Geometry check sheet. Reference: the model listing, model coordinates, mm. A direction names the side the tool comes from. Give positions to 0.01 mm unless a question says otherwise; leave off trailing zeros. Write each loop counter-clockwise with the first axis right and the second up, starting at its lowest first coordinate (ties: lowest second). Pieces come first, ordered by that corner, then holes. Notation, with made-up numbers: (28, 52.5) -> (63, 52.5) arc R22 cw to (63, 69.5) -> close; hole circle Ø10 at (54.5, 88). An arc over 180 degrees is marked (long way). One line per item, written item: value.
from build123d import *

# Parameters (mm, degrees)
FLANGE_PLATE_DEPTH       = 20
OBROUND_NECK_BOSS_DEPTH  = 60
NECK_POCKET_DEPTH        = 30
THROUGH_OPENING_SKETCH_R = 7.5
THROUGH_OPENING_DEPTH    = 50
MOUNTING_HOLES_SKETCH_R  = 10
MOUNTING_HOLES_DEPTH     = 20


with BuildPart() as part:
    # Flange Plate Sketch → Flange Plate (new body)
    with BuildSketch(Plane.XY):
        with BuildLine():
            Line((0, 75), (180, 75))
            ThreePointArc((180, 75), (255, 0), (180, -75))
            Line((180, -75), (0, -75))
            ThreePointArc((0, -75), (-75, 0), (0, 75))
        make_face()
    extrude(amount=FLANGE_PLATE_DEPTH)

    # Neck Boss Sketch → Obround Neck Boss (add)
    with BuildSketch(Plane.XY.offset(20)):
        with BuildLine():
            Line((0, 35), (180, 35))
            ThreePointArc((180, 35), (215, 0), (180, -35))
            Line((180, -35), (0, -35))
            ThreePointArc((0, -35), (-35, 0), (0, 35))
        make_face()
    extrude(amount=OBROUND_NECK_BOSS_DEPTH)

    # Neck Pocket Sketch → Neck Pocket (cut)
    with BuildSketch(Plane.XY.offset(80)):
        with BuildLine():
            Line((0, 20), (180, 20))
            ThreePointArc((180, 20), (200, 0), (180, -20))
            Line((180, -20), (0, -20))
            ThreePointArc((0, -20), (-20, 0), (0, 20))
        make_face()
    extrude(amount=-NECK_POCKET_DEPTH, mode=Mode.SUBTRACT)

    # Through Opening Sketch → Through Opening (cut)
    with BuildSketch(Plane.XY.offset(50)):
        Circle(THROUGH_OPENING_SKETCH_R)
        with Locations((180, 0)):
            Circle(THROUGH_OPENING_SKETCH_R)
        with Locations((90, 0)):
            Circle(THROUGH_OPENING_SKETCH_R)
    extrude(amount=-THROUGH_OPENING_DEPTH, mode=Mode.SUBTRACT)

    # Mounting Holes Sketch → Mounting Holes (cut)
    with BuildSketch(Plane.XY.offset(20)):
        with Locations((0, 55)):
            Circle(MOUNTING_HOLES_SKETCH_R)
        with Locations((181.871324801, 55)):
            Circle(MOUNTING_HOLES_SKETCH_R)
        with Locations((181.871324801, -55.713132711)):
            Circle(MOUNTING_HOLES_SKETCH_R)
        with Locations((0, -55.713132711)):
            Circle(MOUNTING_HOLES_SKETCH_R)
        with Locations((90, 55)):
            Circle(MOUNTING_HOLES_SKETCH_R)
        with Locations((90, -55.713132711)):
            Circle(MOUNTING_HOLES_SKETCH_R)
    extrude(amount=-MOUNTING_HOLES_DEPTH, mode=Mode.SUBTRACT)


solid = part.part
1) Sectioned sample at A-A on y = 0. Record the cut outline in (x, z), plus the area to 4 significant figures.
Verdict:
outline: (-75, 0) -> (-7.5, 0) -> (-7.5, 50) -> (-20, 50) -> (-20, 80) -> (-35, 80) -> (-35, 20) -> (-75, 20) -> close; (7.5, 0) -> (82.5, 0) -> (82.5, 50) -> (7.5, 50) -> close; (97.5, 0) -> (172.5, 0) -> (172.5, 50) -> (97.5, 50) -> close; (187.5, 0) -> (255, 0) -> (255, 20) -> (215, 20) -> (215, 80) -> (200, 80) -> (200, 50) -> (187.5, 50) -> close
area: 12,750 mm^2
2) Sectioned sample at D-D on z = 9. Give the number of separate pieces and of enclosed holes in the cut face, plus the area to 3 significant figures.
Verdict:
separate pieces: 1
enclosed holes: 9
area: 42,300 mm^2
3) Scan lines: probe 1 along Y at (x, z) = (90, 6.25); probe 2 along X at (y, z) = (-55, 11.5); probe 3 along Y at (x, z) = (70.5, 71). Record each from-to range of solid material in increasing order.
Verdict:
probe 1: -75 to -65.71, -45.71 to -7.5, 7.5 to 45, 65 to 75
probe 2: -50.99 to -9.97, 9.97 to 80.03, 99.97 to 171.9, 191.85 to 230.99
probe 3: -35 to -20, 20 to 35
4) Sectioned sample at C-C on x = 60. Record the cut outline in (y, z).
Verdict:
outline: (-75, 0) -> (75, 0) -> (75, 20) -> (35, 20) -> (35, 80) -> (20, 80) -> (20, 50) -> (-20, 50) -> (-20, 80) -> (-35, 80) -> (-35, 20) -> (-75, 20) -> close
5) Depth check by flat-ended pin: pin 1 Ø24 at (x, y) = (90, 0) entering from -Z; pin 2 Ø4 at (y, z) = (-5, 52) entering from -X; pin 3 Ø8 at (y, z) = (-25, 31.5) entering from +X; pin 4 Ø2 at (x, y) = (-8, -5) entering from +Z. Enter the tip coordinate at first touch or a pass-through.
Verdict:
pin 1: z = 0
pin 2: x = -34.87
pin 3: x = 208
pin 4: z = 50
6) Mould release check, pull along X, two halves, no side actions. Record for faces 5 (the cylindrical face through (-74.98, -1.65, 9.86)), 6 (the cylindrical face through (-7.493, 0.33, 25.35)), 7 (the flat face through (92, 18, 0)): released by +X, released by -X, zero draft, split by the parting line, or undercut.
Verdict:
face 5: released by -X
face 6: undercut
face 7: zero draft
7) Sectioned sample at B-B on z = 73. Record the cut outline in (x, y), plus the area to 3 significant figures.
Verdict:
outline: (0, -35) -> (180, -35) arc R35 ccw to (180, 35) -> (0, 35) arc R35 ccw to start; hole (0, -20) -> (180, -20) arc R20 ccw to (180, 20) -> (0, 20) arc R20 ccw to start
area: 7,990 mm^2
8) Tool access check on faces 1 (the flat face through (89, 35, 50)), 2 (the flat face through (92, -9, 50)), 3 (the cylindrical face through (214.99, 0.77, 49.58)), 4 (the flat face through (91, -35, 50)). Record the directions out of +Z, -Z, +X, -X, +Y, -Y that give a thin tool (end or side, any length) a straight path to the whole face; none if there is none.
Verdict:
face 1: +Z, +X, -X, +Y
face 2: +Z
face 3: +Z, +X
face 4: +Z, +X, -X, -Y
